from build123d import *

# Parameters (mm, degrees)
SKETCH1_W           = 70
SKETCH1_H           = 70
BOSS_EXTRUDE1_DEPTH = 30
FILLET2_R           = 10
SKETCH3_R           = 3.5
CUT_EXTRUDE1_DEPTH  = 60
SKETCH4_R           = 22.5
BOSS_EXTRUDE3_DEPTH = 6
SKETCH5_R           = 6
BOSS_EXTRUDE4_DEPTH = 35
CHAMFER1_SIZE       = 1
CHAMFER2_SIZE       = 1
CIRPATTERN1_COUNT   = 4
SKETCH6_R           = 35
BOSS_EXTRUDE5_DEPTH = 50
FILLET3_R           = 10


with BuildPart() as part:
    # Sketch1 → Boss-Extrude1 (new body)
    with BuildSketch(Plane.XY):
        Rectangle(SKETCH1_W, SKETCH1_H)
    extrude(amount=BOSS_EXTRUDE1_DEPTH)

    # Fillet2
    fillet2_edges = [part.edges().sort_by_distance(p)[0] for p in [
        (-35, 35, 15),
        (35, 35, 15),
        (35, -35, 15),
        (-35, -35, 15),
    ]]
    fillet(fillet2_edges, radius=FILLET2_R)

    # Sketch3 → Cut-Extrude1 (cut)
    with BuildSketch(Plane.XY.offset(30)):
        with Locations((-28.284271247, 28.284271247)):
            Circle(SKETCH3_R)
    cut_extrude1 = extrude(amount=-CUT_EXTRUDE1_DEPTH, mode=Mode.SUBTRACT)

    # Sketch4 → Boss-Extrude3 (add)
    with BuildSketch(Plane(origin=(0, 0, 0), x_dir=(-1, 0, 0), z_dir=(0, 0, -1))):
        with Locations(Location((0, 0, 0), (0, 0, 180))):
            Circle(SKETCH4_R)
    extrude(amount=BOSS_EXTRUDE3_DEPTH)

    # Sketch5 → Boss-Extrude4 (add)
    with BuildSketch(Plane(origin=(0, 0, -6), x_dir=(-1, 0, 0), z_dir=(0, 0, -1))):
        Circle(SKETCH5_R)
    extrude(amount=BOSS_EXTRUDE4_DEPTH)

    # Chamfer1
    chamfer1_edges = [part.edges().sort_by_distance(p)[0] for p in [
        (6, 0, -41),
    ]]
    chamfer(chamfer1_edges, length=CHAMFER1_SIZE)

    # Chamfer2
    chamfer2_edges = [part.edges().sort_by_distance(p)[0] for p in [
        (-22.5, 0, -6),
    ]]
    chamfer(chamfer2_edges, length=CHAMFER2_SIZE)

    # CirPattern1: Cut-Extrude1 ×4 about axis
    cirpattern1_axis = Axis((0, 0, 0), (0, 0, 1))
    for i in range(1, CIRPATTERN1_COUNT):
        add(cut_extrude1.rotate(cirpattern1_axis, i * 360 / CIRPATTERN1_COUNT), mode=Mode.SUBTRACT)

    # Sketch6 → Boss-Extrude5 (add)
    with BuildSketch(Plane.XY.offset(30)):
        Circle(SKETCH6_R)
    extrude(amount=BOSS_EXTRUDE5_DEPTH)

    # Fillet3
    fillet3_edges = [part.edges().sort_by_distance(p)[0] for p in [
        (-35, 0, 80),
    ]]
    fillet(fillet3_edges, radius=FILLET3_R)


solid = part.part
Model file for the job. Use its own axes, mm. A direction names the side the tool comes from. Coordinates: 2 decimals unless noted, no trailing zeros. Write each loop counter-clockwise with the first axis right and the second up, starting at its lowest first coordinate (ties: lowest second). Pieces come first, ordered by that corner, then holes. Notation, with made-up numbers: (-18, 65) - (18, 65) arc R27 ccw to (18, 93) - close; hole circle Ø3 at (22.25, -32.75). An arc over 180 degrees is marked (long way). Write each question's results on one line, items separated by ' | '. Start each with the question number.
1) Mould opens along X. For faces 5 (the face through (-29.043, 24.867, 15.21)), 6 (the face through (0, 0, -41)), 7 (the face through (31.99, -32.15, 15.21)) say: pulls with the +X half, pulls with the -X half, needs draft (parallel to the pull), parting line crosses it, or undercut.
2) Cut at B-B (x = 27). Count the separate pieces of the cut face and the enclosed holes in it, then the cut area to 3 significant figures.
3) Cut at C-C (z = -8). Write the cut outline in (x, y).
4) 3-axis set-ups, long thin cutter, end or side, ignore diameter. For faces 1 (the face through (25, -25, 30)), 2 (the face through (-25, -25, 30)), 3 (the face through (-24, 27, 30)), 4 (the face through (4.5, 4.5, -6)): which of +Z, -Z, +X, -X, +Y, -Y reach the whole face in a straight line?
5) Flat gauge pins, fed straight in: P1, Ø8, axis at x = -25.5, y = 1.5, coming from the -Z side; P2, Ø9, axis at x = -28.28, y = -28.28, coming from the -Z side; P3, Ø4, axis at y = -17.5, z = -5, coming from the +X side; P4, Ø12, axis at x = -16, z = 33.5, coming from the -Y side. Where does each tip first touch, or does it go through?
6) Cut at D-D (z = 41). Write the cut outline in (x, y).
7) Probe line 1 along Y through (x, z) = (-31.5, 15.5); line 2 along Z through (x, y) = (-10.5, 7); line 3 along Y through (x, z) = (16.5, 32.5). List the from-to ranges inside material, lowest first. Write a range as from..to.
8) Cut at A-A (z = 7.5). Write the cut outline in (x, y), then the cut area to 3 significant figures.
Returned:
1) face 5: undercut | face 6: needs draft | face 7: pulls with the +X half
2) separate pieces: 3 | enclosed holes: 0 | area: 3,840 mm^2
3) outline: circle Ø12 at (0, 0)
4) face 1: +Z, +X, -Y | face 2: +Z, -X, -Y | face 3: +Z, -X, +Y | face 4: -Z
5) P1: z = -5.96 | P2: z = 0 | P3: x = 16.31 | P4: y = -35
6) outline: circle Ø70 at (0, 0)
7) line 1: -32.6..-29.67, -26.9..26.9, 29.67..32.6 | line 2: -6..80 | line 3: -30.87..30.87
8) outline: (-35, -25) arc R10 ccw to (-25, -35) - (25, -35) arc R10 ccw to (35, -25) - (35, 25) arc R10 ccw to (25, 35) - (-25, 35) arc R10 ccw to (-35, 25) - close; hole circle Ø7 at (-28.28, -28.28); hole circle Ø7 at (-28.28, 28.28); hole circle Ø7 at (28.28, -28.28); hole circle Ø7 at (28.28, 28.28) | area: 4,660 mm^2
